Part model, mm, in its own coordinate system. Round coordinates to 2 decimals unless told otherwise and drop trailing zeros. Loops run counter-clockwise (first coordinate to the right, second up) from the corner with the lowest first, then second, coordinate; pieces in that order, holes last. Notation, with made-up numbers: (7, 24) - (65, 24) arc R12 ccw to (65, 33) - close; hole circle Ø1 at (24, 84). An arc over 180 degrees is marked (long way). Write each question's results on one line, items separated by ' | '. Start each with the question number.
(1) Cut at B-B, the plane z = 57. List the corners of the cut face in (x, y), then the cut area to 3 significant figures.
(2) Cut at A-A, the plane y = -23. List the corners of the cut face in (x, z).
(3) Drill centre lines: L1, parallel to X at y = 5, z = 152.5; L2, parallel to Y at x = -10.5, z = -78. Where is each one in solid material? Low to high.
(4) Flat gauge pins, fed straight in: P1, Ø3, axis at x = -11, z = 92.5, coming from the +Y side; P2, Ø12, axis at x = 11.5, y = 2, coming from the +Z side. Where does each tip first touch, or does it go through?
(5) Cut at C-C, the plane x = -2. List the corners of the cut face in (y, z), then the cut area to 3 significant figures.
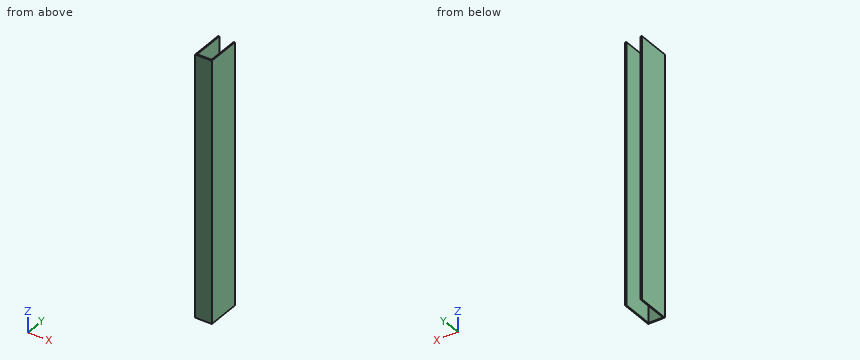
from build123d import *

# Parameters (mm, degrees)
SKETCH_1_W      = 30
SKETCH_1_H      = 60
EXTRUDE_1_DEPTH = 235
SHELL_1_T       = -2


with BuildPart() as part:
    # 草图1 → 凸台-拉伸1 (new, symmetric)
    with BuildSketch(Plane.XY):
        Rectangle(SKETCH_1_W, SKETCH_1_H)
    extrude(amount=EXTRUDE_1_DEPTH, both=True)

    # 抽壳1
    shell_1_openings = [part.faces().sort_by_distance(p)[0] for p in [
        (0, 0, 235),
        (0, 0, -235),
        (0, 30, 0),
    ]]
    offset(amount=SHELL_1_T, openings=shell_1_openings, kind=Kind.INTERSECTION)


solid = part.part
A:
1) outline: (-15, -30) - (15, -30) - (15, 30) - (13, 30) - (13, -28) - (-13, -28) - (-13, 30) - (-15, 30) - close | area: 292 mm2
2) outline: (-15, -235) - (-13, -235) - (-13, 235) - (-15, 235) - close; (13, -235) - (15, -235) - (15, 235) - (13, 235) - close
3) L1: -15 to -13, 13 to 15 | L2: -30 to -28
4) P1: y = -28 | P2: z = 235
5) outline: (-30, -235) - (-28, -235) - (-28, 235) - (-30, 235) - close | area: 940 mm2
